Input: dimensioned drawing with shaded views. Units: mm. Origin: part minimum x, y, z. A direction names the side the tool comes from. Coordinates: 2 decimals unless noted, no trailing zeros. Write each loop counter-clockwise with the first axis right and the second up, starting at its lowest first coordinate (ties: lowest second). Pieces come first, ordered by that corner, then holes. Notation, with made-up numbers: M 37.5,-25 L 85.5,-25 A13 ccw 85.5,-3 Z; hole C 26.25,82 d10. An arc over 180 degrees is marked long. Write each question's results on one line, items separated by ' | '. Start each with the question number.
1. Set-up query: the marked faces 1 and 2. Return all of +Z, -Z, +X, -X, +Y, -Y with unobstructed straight access to the full face (end or side cutting, diameter ignored); none if empty.
2. Section query C-C, the plane x = 34.5. Output: boundary loops of the cut face in (y, z), and give its area (3 significant figures).
3. Section query A-A, the plane y = 15.5. Output: boundary loops of the cut face in (x, z).
4. Section query B-B, the plane x = 10. Output: boundary loops of the cut face in (y, z), and give its area (3 significant figures).
5. Section query D-D, the plane z = 13. Output: boundary loops of the cut face in (x, y).
6. Ray query, probe 1 along Z at (x, y) = (10, 3.5); probe 2 along Y at (x, z) = (5.5, 6.75); probe 3 along Y at (x, z) = (33.5, 10). Return the intervals inside material, ascending.
7. Pull-direction query (X, two-part tool) for the marked faces 3, 4, 5 and 6; classes: +X half, -X half, draft (parallel to the pull), parting line (faces both ways), or undercut.
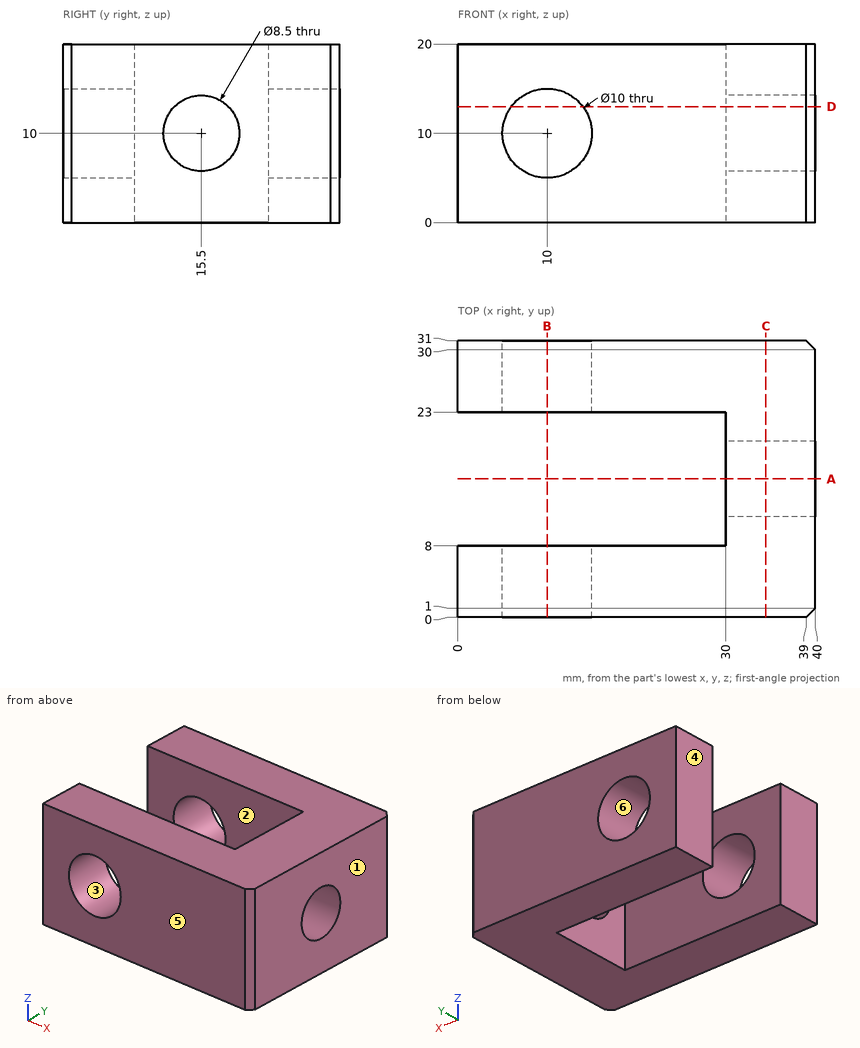
Answer:
1) face 1: +Z, -Z, +X, +Y, -Y | face 2: +Z, -Z, -X
2) outline: M 0,0 L 31,0 L 31,20 L 0,20 Z; hole C 15.5,10 d8.5 | area: 563 mm^2
3) outline: M 30,0 L 40,0 L 40,5.75 L 30,5.75 Z; M 30,14.25 L 40,14.25 L 40,20 L 30,20 Z
4) outline: M 0,0 L 8,0 L 8,5 L 0,5 Z; M 0,15 L 8,15 L 8,20 L 0,20 Z; M 23,0 L 31,0 L 31,5 L 23,5 Z; M 23,15 L 31,15 L 31,20 L 23,20 Z | area: 160 mm^2
5) outline: M 0,0 L 6,0 L 6,8 L 0,8 Z; M 0,23 L 6,23 L 6,31 L 0,31 Z; M 14,0 L 39,0 L 40,1 L 40,12.49 L 30,12.49 L 30,8 L 14,8 Z; M 14,23 L 30,23 L 30,18.51 L 40,18.51 L 40,30 L 39,31 L 14,31 Z
6) probe 1: 0 to 5, 15 to 20 | probe 2: 0 to 8, 23 to 31 | probe 3: 0 to 11.25, 19.75 to 31
7) face 3: undercut | face 4: -X half | face 5: draft | face 6: undercut
